Here's how the part is built. I have some questions about the finished solid (model axes, mm). A direction names the side the tool comes from. Round coordinates to 2 decimals unless told otherwise and drop trailing zeros. Order: outer loops, then holes, each group sorted by start corner. A loop starts at its lowest first (then second) coordinate and runs counter-clockwise, first axis right, second up.
```python
from build123d import *

# Parameters (mm, degrees)
SKETCH_1_W                = 11
SKETCH_1_H                = 23
EXTRUDE_1_DEPTH           = 80
CUT_EXTRUDE_1_DEPTH       = 3.5
HOLE_WIZARD_2_D           = 3.4
HOLE_WIZARD_2_CBORE_D     = 6
HOLE_WIZARD_2_CBORE_DEPTH = 6.9
HOLE_WIZARD_M5_1_D        = 4.2
HOLE_WIZARD_M5_1_DEPTH    = 12.4
HOLE_WIZARD_M5_1_TIP      = 1.2618073
HOLE_WIZARD_M3_1_D        = 2.5
CHAMFER_1_SIZE            = 1


with BuildPart() as part:
    # 草图1 → 凸台-拉伸1 (new body)
    with BuildSketch(Plane(origin=(0, 0, 0), x_dir=(1, 0, 0), z_dir=(0, 1, 0))):
        with Locations((5.5, 11.5)):
            Rectangle(SKETCH_1_W, SKETCH_1_H)
    extrude(amount=EXTRUDE_1_DEPTH)

    # 草图2 → 切除-拉伸1 (cut)
    with BuildSketch(Plane(origin=(11, 0, 0), x_dir=(0, 0, -1), z_dir=(1, 0, 0))):
        with BuildLine():
            Line((23, 80), (14, 80))
            Line((14, 80), (14, 20.5))
            ThreePointArc((14, 20.5), (13.646446609, 19.646446609), (14.5, 20))
            Line((14.5, 20), (23, 20))
            Line((23, 20), (23, 80))
        make_face()
    extrude(amount=-CUT_EXTRUDE_1_DEPTH, mode=Mode.SUBTRACT)

    # 打孔尺寸(%根据)内六角圆柱头螺钉的类型2 (through all)
    with Locations(Plane(origin=(11, 0, 0), x_dir=(0, 0, -1), z_dir=(1, 0, 0))):
        with Locations((4, 20), (4, 30), (19, 30), (19, 20), (4, 60), (4, 70), (19, 60), (19, 70)):
            CounterBoreHole(HOLE_WIZARD_2_D / 2, HOLE_WIZARD_2_CBORE_D / 2, HOLE_WIZARD_2_CBORE_DEPTH)

    # M5 螺纹孔1
    with Locations(Plane(origin=(0, 0, 0), x_dir=(-1, 0, 0), z_dir=(0, -1, 0))):
        with Locations((-5.5, 11.5)):
            Hole(HOLE_WIZARD_M5_1_D / 2, depth=HOLE_WIZARD_M5_1_DEPTH)
            with Locations((0, 0, -(HOLE_WIZARD_M5_1_DEPTH + HOLE_WIZARD_M5_1_TIP / 2))):  # 118° drill point
                Cone(0, HOLE_WIZARD_M5_1_D / 2, HOLE_WIZARD_M5_1_TIP, mode=Mode.SUBTRACT)

    # M3 螺纹孔1 (through all)
    with Locations(Plane(origin=(7.5, 0, 0), x_dir=(0, 0, -1), z_dir=(1, 0, 0))):
        with Locations((19.5, 25), (19.5, 50), (19.5, 75)):
            Hole(HOLE_WIZARD_M3_1_D / 2)

    # 倒角1
    chamfer_1_edges = [part.edges().sort_by_distance(p)[0] for p in [
        (3.75, 80, -23),
        (5.5, 80, 0),
        (5.5, 0, -23),
        (5.5, 0, 0),
    ]]
    chamfer(chamfer_1_edges, length=CHAMFER_1_SIZE)


solid = part.part
```
1. If we section it at B-B, the plane y = 30: Write out the boundary of the cut face in (x, z), and give its area (3 significant figures).
Evaluation:
outline: (0, -23) - (7.5, -23) - (7.5, -22) - (4.1, -22) - (4.1, -20.7) - (0, -20.7) - close; (0, -17.3) - (4.1, -17.3) - (4.1, -16) - (7.5, -16) - (7.5, -14) - (11, -14) - (11, -7) - (4.1, -7) - (4.1, -5.7) - (0, -5.7) - close; (0, -2.3) - (4.1, -2.3) - (4.1, -1) - (11, -1) - (11, 0) - (0, 0) - close
area: 132 mm2
2. If we section it at D-D, the plane x = 1.25: State how many separate pieces and enclosed holes the cut face has, and give its area (3 significant figures).
Evaluation:
separate pieces: 1
enclosed holes: 11
area: 1,750 mm2
3. On a 3-axis mill with a long thin cutter (end or side, diameter ignored), from which of +Z, -Z, +X, -X, +Y, -Y can I reach the whole of each face in a straight line? I mean faces 5 (the flat face through (4.1, 18, -19)), 6 (the flat face through (9, 51, -14)), 7 (the cylindrical face through (5.227, 6.287, -13.582)). Say none if no direction works.
Evaluation:
face 5: +X
face 6: -Z, +X, +Y
face 7: -Y
4. I need wall thicknesses on probe 1 along Y at (x, z) = (3.05, -4); probe 2 along Z at (x, y) = (5.75, 9); probe 3 along X at (y, z) = (66.5, -20). Which ranges of each line are inside material? Lowest first, please.
Evaluation:
probe 1: y = 0 to 18.3, 21.7 to 28.3, 31.7 to 58.3, 61.7 to 68.3, 71.7 to 80
probe 2: z = -23 to -13.59, -9.41 to 0
probe 3: x = 0 to 7.5
5. If we mould it in two halves opening along Y, with no side actions, what happens to faces 1 (the flat face through (4.1, 70, -6)), 2 (the flat face through (5, 80, -12)), 3 (the flat face through (5, 39, 0)), 4 (the conical face through (5.789, 13.443, -11.278))? For each: released by +Y, released by -Y, zero draft, split by the parting line, or undercut.
Evaluation:
face 1: undercut
face 2: released by +Y
face 3: zero draft
face 4: released by -Y
6. I'm going to push flat-ended pins straight in: P1, Ø5, axis at y = 30, z = -18, coming from the +X side; P2, Ø3.5, axis at y = 60, z = -4, coming from the +X side; P3, Ø2.5, axis at y = 60, z = -19, coming from the -X side. Where does each tip first touch, or does it pass through?
Evaluation:
P1: stops at x = 7.5
P2: stops at x = 4.1
P3: passes through
7. If we section it at C-C, the plane x = 10: Write out the boundary of the cut face in (y, z), and give its area (3 significant figures).
Evaluation:
outline: (0, -22) - (1, -23) - (20, -23) - (20, -22) arc R3 cw to (20, -16) - (20, -14.5) arc R0.5 cw (long way) to (20.5, -14) - (80, -14) - (80, -1) - (79, 0) - (1, 0) - (0, -1) - close; hole circle Ø6 at (20, -4); hole circle Ø6 at (30, -4); hole circle Ø6 at (60, -4); hole circle Ø6 at (70, -4)
area: 1,170 mm2
8. If we section it at A-A, the plane y = 50: Write out the boundary of the cut face in (x, z).
Evaluation:
outline: (0, -23) - (7.5, -23) - (7.5, -20.75) - (0, -20.75) - close; (0, -18.25) - (7.5, -18.25) - (7.5, -14) - (11, -14) - (11, 0) - (0, 0) - close
